Geometry: see drawing. Coordinates: mm, zero at the bounding-box minimum. A direction names the side the tool comes from. Round coordinates to 2 decimals unless told otherwise and drop trailing zeros. Write each loop counter-clockwise with the first axis right and the second up, starting at its lowest first coordinate (ties: lowest second). Pieces come first, ordered by that corner, then holes.
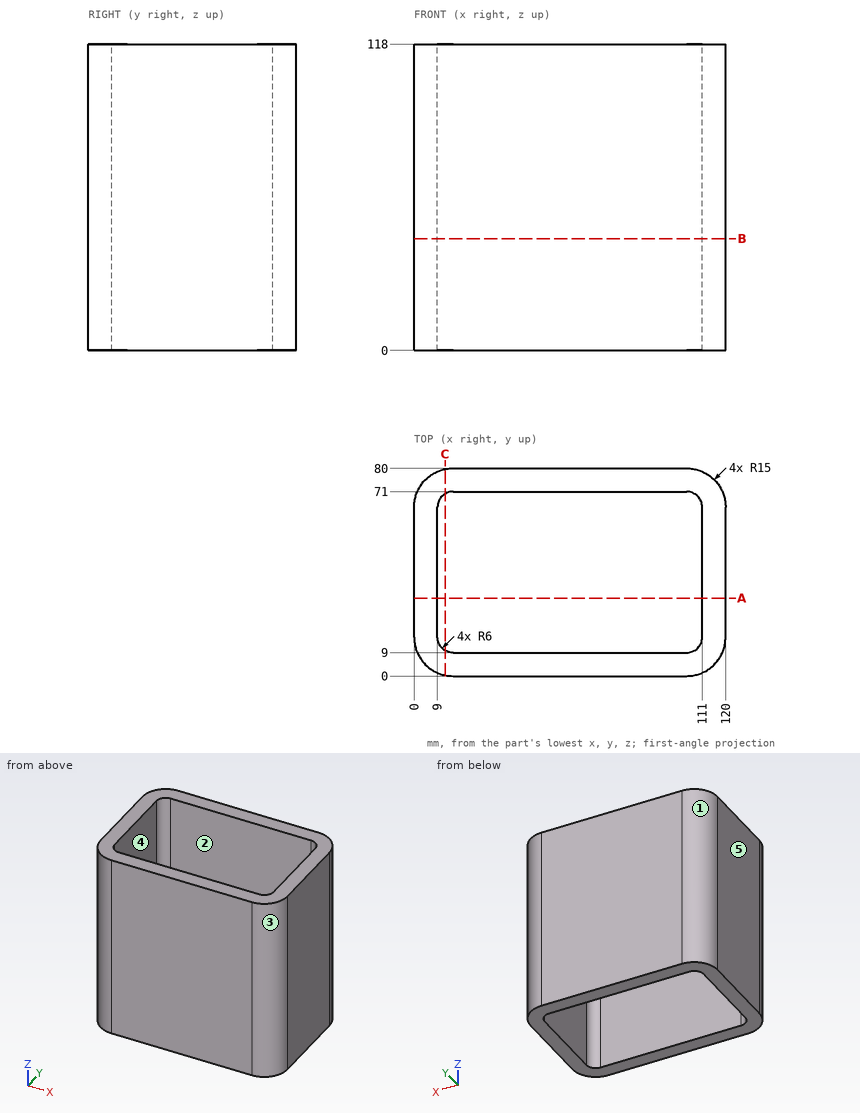
1) Pull-direction query (Y, two-part tool) for the marked faces 1, 2 and 3; classes: released by +Y, released by -Y, zero draft, split by the parting line, or undercut.
Taken from the geometry:
face 1: released by +Y
face 2: undercut
face 3: released by -Y
2) Section query B-B on z = 43. Return the cut outline in (x, y), then the cut area to 3 significant figures.
Taken from the geometry:
outline: (0, 15) arc R15 ccw to (15, 0) - (105, 0) arc R15 ccw to (120, 15) - (120, 65) arc R15 ccw to (105, 80) - (15, 80) arc R15 ccw to (0, 65) - close; hole (9, 15) arc R6 ccw to (15, 9) - (105, 9) arc R6 ccw to (111, 15) - (111, 65) arc R6 ccw to (105, 71) - (15, 71) arc R6 ccw to (9, 65) - close
area: 3,110 mm2
3) Section query C-C on x = 12. Return the cut outline in (y, z), then the cut area to 3 significant figures.
Taken from the geometry:
outline: (0.3, 0) - (9.8, 0) - (9.8, 118) - (0.3, 118) - close; (70.2, 0) - (79.7, 0) - (79.7, 118) - (70.2, 118) - close
area: 2,240 mm2
4) Material intervals for line 1 (Y direction, x = 28, z = 86); line 2 (X direction, y = 34, z = 7); line 3 (X direction, y = 13.5, z = 54), sorted ascending.
Taken from the geometry:
line 1: y = 0 to 9, 71 to 80
line 2: x = 0 to 9, 111 to 120
line 3: x = 0.08 to 9.19, 110.81 to 119.92
5) Contact query for flat-ended pins moving along their axis: P1, Ø12, axis at x = 45.5, y = 20.5, coming from the +Z side; P2, Ø10, axis at x = 106.5, z = 76.5, coming from the +Y side; P3, Ø1.5, axis at y = 67.5, z = 92, coming from the +X side. Output: stop coordinate, or through.
Taken from the geometry:
P1: passes through
P2: stops at y = 80
P3: stops at x = 119.9
6) Reachability of the marked faces 4 and 5 from +Z, -Z, +X, -X, +Y, -Y: full face, straight path, thin tool, end or side. Return the list, or none.
Taken from the geometry:
face 4: +Z, -Z
face 5: +Z, -Z, -X, +Y, -Y
7) Section query A-A on y = 30. Return the cut outline in (x, z), then the cut area to 3 significant figures.
Taken from the geometry:
outline: (0, 0) - (9, 0) - (9, 118) - (0, 118) - close; (111, 0) - (120, 0) - (120, 118) - (111, 118) - close
area: 2,120 mm2
